Could you check a few things on this model? Use its own coordinates, in mm. Face numbers are marked on the shaded views. A direction names the side the tool comes from. Coordinates: 2 decimals unless noted, no trailing zeros. Loops run counter-clockwise (first coordinate to the right, second up) from the corner with the lowest first, then second, coordinate; pieces in that order, holes last. Notation, with made-up numbers: M -10.75,70.5 L 44.25,70.5 A18 cw 44.25,100.5 Z; hole C -39.75,5 d6. An arc over 180 degrees is marked long. Write each question's results on one line, items separated by ' | '.
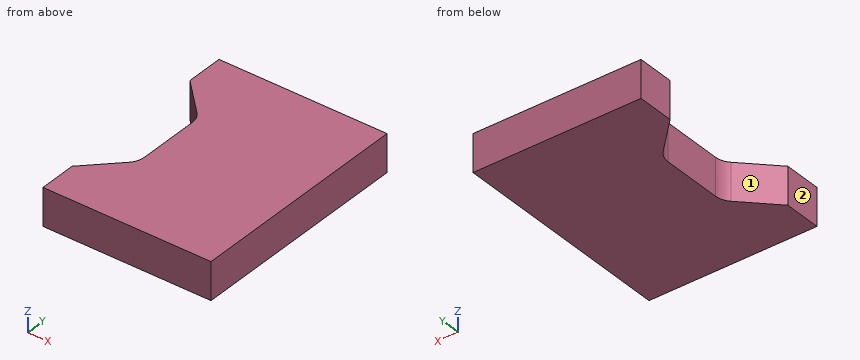
```python
from build123d import *

# Parameters (mm, degrees)
BOSS_EXTRUDE1_DEPTH = 20


with BuildPart() as part:
    # Sketch1 → Boss-Extrude1 (new body)
    with BuildSketch(Plane.XY):
        with BuildLine():
            Line((0, 0), (90, 0))
            Line((90, 0), (90, -121))
            Line((90, -121), (0, -121))
            Line((0, -121), (0, -101))
            Line((0, -101), (17.071067812, -83.928932188))
            ThreePointArc((17.071067812, -83.928932188), (19.238795325, -80.6846987), (20, -76.857864376))
            Line((20, -76.857864376), (20, -44.142135624))
            ThreePointArc((20, -44.142135624), (19.238795325, -40.3153013), (17.071067812, -37.071067812))
            Line((17.071067812, -37.071067812), (0, -20))
            Line((0, -20), (0, 0))
        make_face()
    extrude(amount=BOSS_EXTRUDE1_DEPTH)


solid = part.part
```
(1) Imagine slicing it at B-B, the plane z = 15.75. List the corners of the cut face in (x, y) for me.
Reported:
outline: M 0,-121 L 90,-121 L 90,0 L 0,0 L 0,-20 L 17.07,-37.07 A10 cw 20,-44.14 L 20,-76.86 A10 cw 17.07,-83.93 L 0,-101 Z
(2) Which directions (+Z, -Z, +X, -X, +Y, -Y) give clear straight access to the entire face, cutting with the end or side of a thin tool? Please do the marked faces 1 and 2.
Reported:
face 1: +Z, -Z, -X | face 2: +Z, -Z, -X, +Y, -Y
(3) Will these pins go through, and if not, where does the flat tip stop? P1, Ø12, axis at y = -28.5, z = 6, coming from the -X side; P2, Ø2, axis at y = -65.5, z = 12.5, coming from the -X side; P3, Ø2, axis at x = 76.5, z = 11, coming from the +Y side.
Reported:
P1: stops at x = 2.5 | P2: stops at x = 20 | P3: stops at y = 0
(4) Imagine slicing it at D-D, the plane y = -95.5. List the corners of the cut face in (x, z) for me, and give its area (3 significant figures).
Reported:
outline: M 5.5,0 L 90,0 L 90,20 L 5.5,20 Z | area: 1,690 mm2
(5) Please list where these lines run through material, in increasing order: probe 1 along X at (y, z) = (-55.5, 15.25); probe 2 along Y at (x, z) = (5, 8.25); probe 3 along Y at (x, z) = (11, 9.25). Write a range as from..to.
Reported:
probe 1: x = 20..90 | probe 2: y = -121..-96, -25..0 | probe 3: y = -121..-90, -31..0
(6) Imagine slicing it at A-A, the plane x = 7. List the corners of the cut face in (y, z) for me.
Reported:
outline: M -121,0 L -94,0 L -94,20 L -121,20 Z; M -27,0 L 0,0 L 0,20 L -27,20 Z
(7) Imagine slicing it at C-C, the plane y = -23. List the corners of the cut face in (x, z) for me.
Reported:
outline: M 3,0 L 90,0 L 90,20 L 3,20 Z
